from build123d import *

# Parameters (mm, degrees)
SKETCH1_W                                         = 150
SKETCH1_H                                         = 80
BOSS_EXTRUDE1_DEPTH                               = 14
HOLE_SIZE_BY_SOCKET_HEAD_CAP_SCREW_TY_D           = 9
HOLE_SIZE_BY_SOCKET_HEAD_CAP_SCREW_TY_CBORE_D     = 15
HOLE_SIZE_BY_SOCKET_HEAD_CAP_SCREW_TY_CBORE_DEPTH = 9
F_9_0_9_DIAMETER_HOLE1_D                          = 9


with BuildPart() as part:
    # Sketch1 → Boss-Extrude1 (new body)
    with BuildSketch(Plane(origin=(0, 0, 0), x_dir=(1, 0, 0), z_dir=(0, 1, 0))):
        with Locations((75, 40)):
            Rectangle(SKETCH1_W, SKETCH1_H)
    extrude(amount=BOSS_EXTRUDE1_DEPTH)

    # Hole size (% by) socket head cap screw type1 (through all)
    with Locations(Plane(origin=(0, 14, 0), x_dir=(-1, 0, 0), z_dir=(0, 1, 0))):
        with Locations((-52.5, -68.5), (-52.5, -11.5), (-97.5, -11.5), (-97.5, -68.5)):
            CounterBoreHole(HOLE_SIZE_BY_SOCKET_HEAD_CAP_SCREW_TY_D / 2, HOLE_SIZE_BY_SOCKET_HEAD_CAP_SCREW_TY_CBORE_D / 2, HOLE_SIZE_BY_SOCKET_HEAD_CAP_SCREW_TY_CBORE_DEPTH)

    # Ø9.0 (9) Diameter Hole1 (through all)
    with Locations(Plane(origin=(0, 14, 0), x_dir=(-1, 0, 0), z_dir=(0, 1, 0))):
        with Locations((-15, -65), (-15, -15), (-135, -15), (-135, -65)):
            Hole(F_9_0_9_DIAMETER_HOLE1_D / 2)


solid = part.part
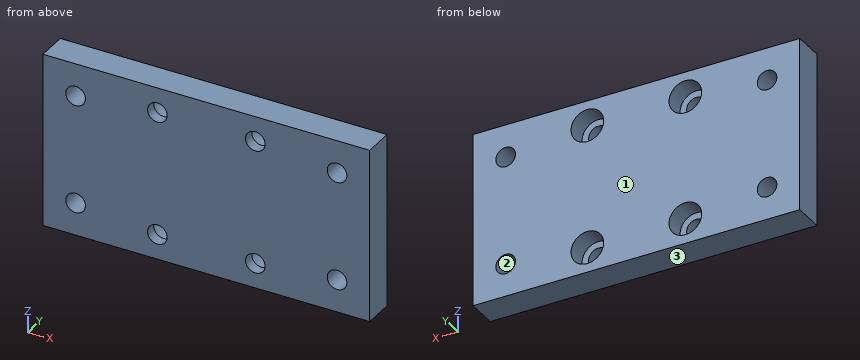
Source: CAD feature listing. Evaluate the final solid. Frame: model axes, mm. Face numbers are marked on the shaded views. Give positions to 0.01 mm unless a question says otherwise; leave off trailing zeros. Write each loop counter-clockwise with the first axis right and the second up, starting at its lowest first coordinate (ties: lowest second). Pieces come first, ordered by that corner, then holes. Notation, with made-up numbers: (75, 70) - (101, 70) arc R24 ccw to (101, 82) - close; hole circle Ø8 at (-1.5, 58.25). An arc over 180 degrees is marked (long way). Write item = value, one per line. Start each with the question number.
Q1. Pin query (flat end, axial travel): pin 1 Ø7.5 at (x, z) = (96, -70.5) entering from +Y. Return the tip coordinate at first contact, or that it passes through.
Q2. Cut plane B-B, the plane y = 7.25. Give the number of separate pieces and of enclosed holes in the cut face, then the cut area to 3 significant figures.
Q3. Material intervals for probe 1 along Z at (x, y) = (15, 6.25); probe 2 along X at (y, z) = (7.75, -16); probe 3 along Z at (x, y) = (18, 7.5), sorted ascending.
Q4. Draft query along Z for the marked faces 1, 2 and 3. Return one class per face: +Z half, -Z half, draft (parallel to the pull), parting line (faces both ways), or undercut.
Q5. Cut plane D-D, the plane x = 135. Return loops of the section in (y, z), then the cut area to 3 significant figures.
Q6. Cut plane A-A, the plane x = 97.5. Return loops of the section in (y, z).
Q7. Cut plane C-C, the plane z = -13. Return loops of the section in (x, y), then the cut area to 3 significant figures.
Computed values:
q1.pin_1 = 5
q2.separate_pieces = 1
q2.enclosed_holes = 8
q2.area = 11,000 mm²
q3.probe_1 = -80 to -69.5, -60.5 to -19.5, -10.5 to 0
q3.probe_2 = 0 to 10.61, 19.39 to 46.5, 58.5 to 91.5, 103.5 to 130.61, 139.39 to 150
q3.probe_3 = -80 to -68.35, -61.65 to -18.35, -11.65 to 0
q4.face_1 = draft
q4.face_2 = undercut
q4.face_3 = -Z half
q5.outline = (0, -80) - (14, -80) - (14, -69.5) - (0, -69.5) - close; (0, -60.5) - (14, -60.5) - (14, -19.5) - (0, -19.5) - close; (0, -10.5) - (14, -10.5) - (14, 0) - (0, 0) - close
q5.area = 868 mm²
q6.outline = (0, -80) - (14, -80) - (14, -76) - (5, -76) - (5, -73) - (0, -73) - close; (0, -64) - (5, -64) - (5, -61) - (14, -61) - (14, -19) - (5, -19) - (5, -16) - (0, -16) - close; (0, -7) - (5, -7) - (5, -4) - (14, -4) - (14, 0) - (0, 0) - close
q7.outline = (0, 0) - (10.97, 0) - (10.97, 14) - (0, 14) - close; (19.03, 0) - (48.26, 0) - (48.26, 5) - (45.15, 5) - (45.15, 14) - (19.03, 14) - close; (56.74, 0) - (93.26, 0) - (93.26, 5) - (90.15, 5) - (90.15, 14) - (59.85, 14) - (59.85, 5) - (56.74, 5) - close; (101.74, 0) - (130.97, 0) - (130.97, 14) - (104.85, 14) - (104.85, 5) - (101.74, 5) - close; (139.03, 0) - (150, 0) - (150, 14) - (139.03, 14) - close
q7.area = 1,520 mm²
